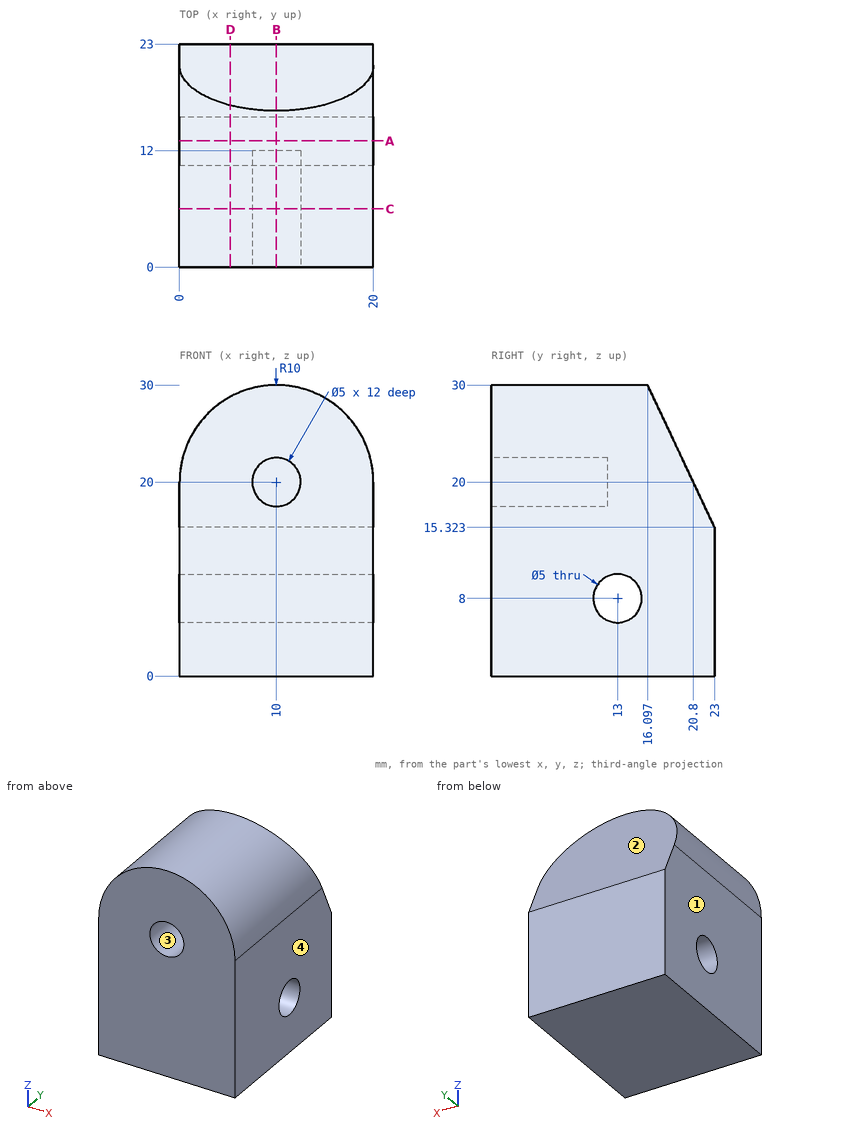
Job drawing, mm, ordinate dimensions from the low corner. One solid piece. Give positions to 0.01 mm unless a question says otherwise; leave off trailing zeros. Write each loop counter-clockwise with the first axis right and the second up, starting at its lowest first coordinate (ties: lowest second). Pieces come first, ordered by that corner, then holes. Notation, with made-up numbers: (-30.75, 14.25) - (-3.75, 14.25) arc R9 cw to (-3.75, 28.25) - close; hole circle Ø7 at (79, -29). An arc over 180 degrees is marked (long way). Use one line per item in the form item = value. Start each with the question number.
1. Band-saw the part on B-B on x = 10. Write the cut outline in (y, z).
2. Band-saw the part on A-A on y = 13. Write the cut outline in (x, z).
3. Two-plate mould, pull along X, no slides. Class the marked faces 1, 2, 3 and 4: released by +X, released by -X, zero draft, split by the parting line, or undercut.
4. Band-saw the part on D-D on x = 5.25. Write the cut outline in (y, z).
5. Drop flat-ended pins along their axis: pin 1 Ø4 at (y, z) = (13, 8) entering from -X; pin 2 Ø4 at (x, y) = (14.5, 10) entering from +Z; pin 3 Ø6 at (x, z) = (10, 20) entering from +Y. Give the stop position or say it passes through.
6. Band-saw the part on C-C on y = 6. Write the cut outline in (x, z).
7. Probe line 1 (X direction, y = 9, z = 20); line 2 (Y direction, x = 9, z = 6.25) (1 decimal); line 3 (X direction, y = 5, z = 19.5). List the from-to ranges inside material, lowest first. Write a range as [from, to].
Conclusion:
q1.outline = (0, 0) - (23, 0) - (23, 15.32) - (16.1, 30) - (0, 30) - (0, 22.5) - (12, 22.5) - (12, 17.5) - (0, 17.5) - close; hole circle Ø5 at (13, 8)
q2.outline = (0, 0) - (20, 0) - (20, 5.5) - (0, 5.5) - close; (0, 10.5) - (20, 10.5) - (20, 20) arc R10 ccw to (0, 20) - close
q3.face_1 = released by -X
q3.face_2 = zero draft
q3.face_3 = undercut
q3.face_4 = released by +X
q4.outline = (0, 0) - (23, 0) - (23, 15.32) - (16.66, 28.8) - (0, 28.8) - close; hole circle Ø5 at (13, 8)
q5.pin_1 = through
q5.pin_2 = 29.68
q5.pin_3 = 22.21
q6.outline = (0, 0) - (20, 0) - (20, 20) arc R10 ccw to (0, 20) - close; hole circle Ø5 at (10, 20)
q7.line_1 = [0, 7.5], [12.5, 20]
q7.line_2 = [0, 11.2], [14.8, 23]
q7.line_3 = [0, 7.55], [12.45, 20]
